The model under review builds one solid part; all positions refer to its coordinate system, in mm. A direction names the side the tool comes from. Coordinates: 2 decimals unless noted, no trailing zeros. Order: outer loops, then holes, each group sorted by start corner. A loop starts at its lowest first (then second) coordinate and runs counter-clockwise, first axis right, second up. Notation, with made-up numbers: (-24.5, -21.5) -> (-11.5, -21.5) arc R14 cw to (-11.5, 1.5) -> close; hole circle Ø6 at (41.25, 18.5). An arc over 180 degrees is marked (long way). Use one line per item in the form item = value. Start each with the question number.
(1) Take a section at C-C (y = 0.85). State the section outline as (x, z) points, then the cut area to 3 significant figures.
(2) Take a section at A-A (x = -50). State the section outline as (y, z) points.
(3) Mouldability with a two-part tool opening along X and no side actions: class faces 1 (the cylindrical face through (-79.14, 2.03, 79.1)), 2 (the flat face through (-41, 2, 0)), 3 (the cylindrical face through (-70, 2, 70)) as +X half, -X half, draft (parallel to the pull), parting line (faces both ways), or undercut.
(4) Take a section at B-B (z = 20). State the section outline as (x, y) points.
(5) For faces 4 (the cylindrical face through (-0.9, 2.03, 0.86)), 5 (the flat face through (-45, 2, 60)), list the 3-axis set-ups (+Z, -Z, +X, -X, +Y, -Y) from which the entire face can be reached by the end or side of a thin tool; tool diameter is ignored.
(6) Wall thickness on line 1 along X through (y, z) = (2.55, 58.5); line 2 along X through (y, z) = (3.05, 20); line 3 along X through (y, z) = (3, 10): over which ranges is each line inside the solid? List them lowest first.
(7) Take a section at D-D (z = 69). State the section outline as (x, y) points.
```python
from build123d import *

# Parameters (mm, degrees)
SKETCH1_W           = 80
SKETCH1_H           = 80
SKETCH1_R           = 9
BOSS_EXTRUDE1_DEPTH = 4
FILLET1_R           = 3


with BuildPart() as part:
    # Sketch1 → Boss-Extrude1 (new body)
    with BuildSketch(Plane(origin=(0, 0, 0), x_dir=(1, 0, 0), z_dir=(0, 1, 0))):
        with Locations((-40, -40)):
            Rectangle(SKETCH1_W, SKETCH1_H)
        with Locations(Location((-60, -20, 0), (0, 0, 270))):
            Circle(SKETCH1_R, mode=Mode.SUBTRACT)
        with BuildLine():
            Line((-25, -5), (-15, -5))
            ThreePointArc((-15, -5), (-10, -10), (-15, -15))
            Line((-15, -15), (-25, -15))
            ThreePointArc((-25, -15), (-30, -10), (-25, -5))
        make_face(mode=Mode.SUBTRACT)
        with BuildLine():
            Line((-65, -55), (-65, -65))
            ThreePointArc((-65, -65), (-70, -70), (-75, -65))
            Line((-75, -65), (-75, -55))
            ThreePointArc((-75, -55), (-70, -50), (-65, -55))
        make_face(mode=Mode.SUBTRACT)
        with BuildLine():
            Line((-45, -55), (-45, -65))
            ThreePointArc((-45, -65), (-50, -70), (-55, -65))
            Line((-55, -65), (-55, -55))
            ThreePointArc((-55, -55), (-50, -50), (-45, -55))
        make_face(mode=Mode.SUBTRACT)
    extrude(amount=BOSS_EXTRUDE1_DEPTH)

    # Fillet1
    fillet1_edges = [part.edges().sort_by_distance(p)[0] for p in [
        (0, 2, 80),
        (-80, 2, 80),
        (-80, 2, 0),
        (0, 2, 0),
    ]]
    fillet(fillet1_edges, radius=FILLET1_R)


solid = part.part
```
Findings:
q1.outline = (-80, 3) arc R3 ccw to (-77, 0) -> (-3, 0) arc R3 ccw to (0, 3) -> (0, 77) arc R3 ccw to (-3, 80) -> (-77, 80) arc R3 ccw to (-80, 77) -> close; hole (-75, 55) arc R5 ccw to (-65, 55) -> (-65, 65) arc R5 ccw to (-75, 65) -> close; hole circle Ø18 at (-60, 20); hole (-55, 55) arc R5 ccw to (-45, 55) -> (-45, 65) arc R5 ccw to (-55, 65) -> close; hole (-25, 5) -> (-15, 5) arc R5 ccw to (-15, 15) -> (-25, 15) arc R5 ccw to start
q1.area = 5,600 mm²
q2.outline = (0, 0) -> (4, 0) -> (4, 50) -> (0, 50) -> close; (0, 70) -> (4, 70) -> (4, 80) -> (0, 80) -> close
q3.face_1 = -X half
q3.face_2 = draft
q3.face_3 = undercut
q4.outline = (-80, 0) -> (-69, 0) -> (-69, 4) -> (-80, 4) -> close; (-51, 0) -> (0, 0) -> (0, 4) -> (-51, 4) -> close
q5.face_4 = -Z, +X, +Y, -Y
q5.face_5 = +Y, -Y
q6.line_1 = -80 to -75, -65 to -55, -45 to 0
q6.line_2 = -80 to -69, -51 to 0
q6.line_3 = -80 to -30, -10 to 0
q7.outline = (-80, 0) -> (-73, 0) -> (-73, 4) -> (-80, 4) -> close; (-67, 0) -> (-53, 0) -> (-53, 4) -> (-67, 4) -> close; (-47, 0) -> (0, 0) -> (0, 4) -> (-47, 4) -> close
